Part print with two shaded views. Sizes in mm from the minimum x, y, z corner. A direction names the side the tool comes from. Coordinates: 2 decimals unless noted, no trailing zeros. Loops run counter-clockwise (first coordinate to the right, second up) from the corner with the lowest first, then second, coordinate; pieces in that order, holes last. Notation, with made-up numbers: (59, 57.25) -> (64, 57.25) arc R27 cw to (64, 94.25) -> close; hole circle Ø6 at (-20, -12). An arc over 180 degrees is marked (long way). Return JSON: item names as keys, results as strings. Group by question number.
(1) Saw through at C-C on z = 3.25. Write the cut outline in (x, y), then the cut area to 3 significant figures.
(2) Saw through at A-A on y = 10. Write the cut outline in (x, z), then the cut area to 3 significant figures.
(3) Flat gauge pins, fed straight in: pin 1 Ø3 at (y, z) = (3, 7.5) entering from -X; pin 2 Ø2 at (y, z) = (14.5, 5.5) entering from -X; pin 3 Ø3 at (y, z) = (10.5, 3) entering from -X. Where does each tip first touch, or does it go through?
(4) Saw through at D-D on y = 16.25. Write the cut outline in (x, z), then the cut area to 3 significant figures.
(5) Probe L1, parallel to Y at x = 10, z = 2.75; L2, parallel to Z at x = 14.25, y = 1.75; L3, parallel to X at y = 7.75, z = 3. List the from-to ranges inside material, lowest first.
(6) Mould opens along X. For the marked faces 3, 4 and 5 say: pulls with the +X half, pulls with the -X half, needs draft (parallel to the pull), parting line crosses it, or undercut.
(7) Tool access for the marked faces 1 and 2: list every direction of +Z, -Z, +X, -X, +Y, -Y with a clear straight run to the whole face (end or side of a thin tool).
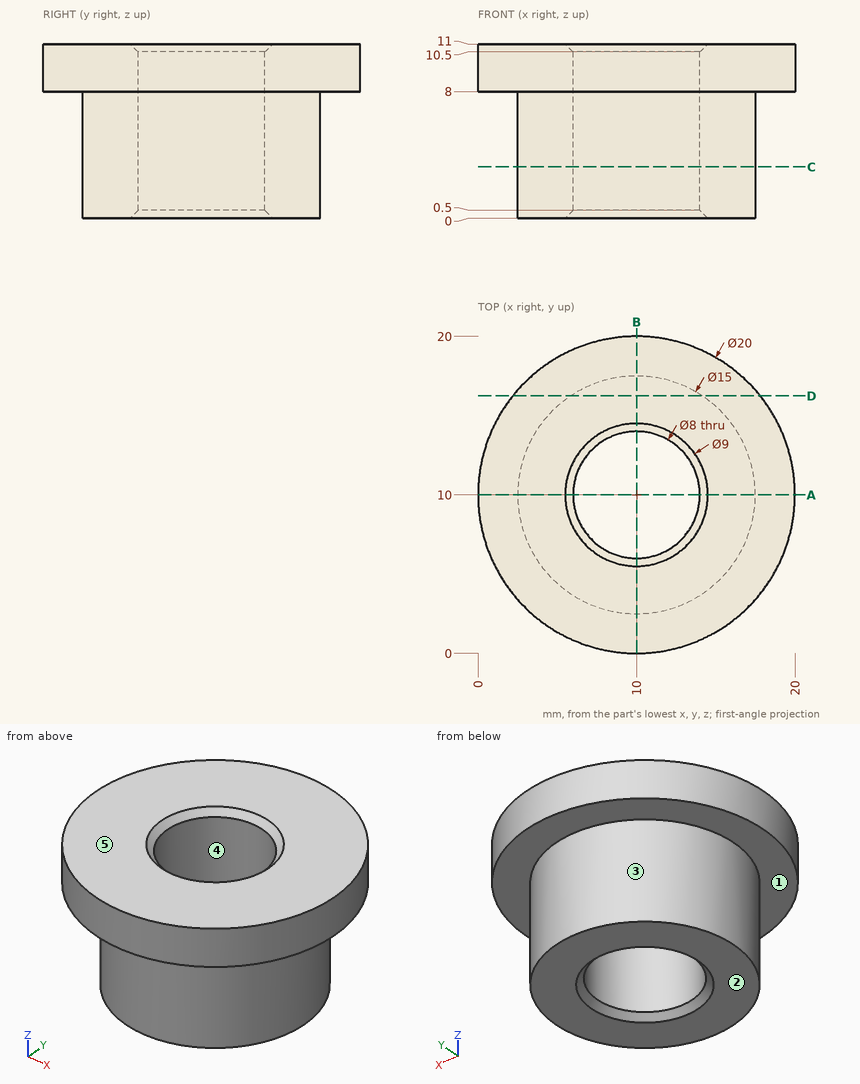
Geometry results:
{
 "1": {"outline": "circle Ø15 at (10, 10); hole circle Ø8 at (10, 10)", "area": "126 mm²"},
 "2": {"outline": "(0, 8) -> (2.5, 8) -> (2.5, 0) -> (5.5, 0) -> (6, 0.5) -> (6, 10.5) -> (5.5, 11) -> (0, 11) -> close; (14, 0.5) -> (14.5, 0) -> (17.5, 0) -> (17.5, 8) -> (20, 8) -> (20, 11) -> (14.5, 11) -> (14, 10.5) -> close", "area": "91.5 mm²"},
 "3": {"pin 1": "x = 1.71", "pin 2": "x = 3.37", "pin 3": "x = 2.5"},
 "4": {"outline": "(2.19, 8) -> (5.85, 8) -> (5.85, 0) -> (14.15, 0) -> (14.15, 8) -> (17.81, 8) -> (17.81, 11) -> (2.19, 11) -> close", "area": "113 mm²"},
 "5": {"L1": "2.5 to 6, 14 to 17.5", "L2": "8 to 11", "L3": "2.85 to 6.69, 13.31 to 17.15"},
 "6": {"face 3": "parting line crosses it", "face 4": "undercut", "face 5": "needs draft"},
 "7": {"face 1": "-Z", "face 2": "-Z, +X, -X, +Y, -Y"}
}
